```python
from build123d import *

# Parameters (mm, degrees)
BASE_PLATE_DEPTH       = 1
RIM_WALL_DEPTH         = 2
SIDE_GROOVE_A_SKETCH_W = 1
SIDE_GROOVE_A_SKETCH_H = 1
SIDE_GROOVE_A_DEPTH    = 40
SIDE_GROOVE_B_SKETCH_W = 1
SIDE_GROOVE_B_SKETCH_H = 1
SIDE_GROOVE_B_DEPTH    = 40


with BuildPart() as part:
    # Base Plate Sketch → Base Plate (new body)
    with BuildSketch(Plane(origin=(0, 0, 0), x_dir=(1, 0, 0), z_dir=(0, 1, 0))):
        with BuildLine():
            Line((-10.246950766, 12), (10.246950766, 12))
            ThreePointArc((10.246950766, 12), (12.001066805, 11.594868137), (13.399858694, 10.461538462))
            ThreePointArc((13.399858694, 10.461538462), (17, 0), (13.399858694, -10.461538462))
            ThreePointArc((13.399858694, -10.461538462), (12.001066805, -11.594868137), (10.246950766, -12))
            Line((10.246950766, -12), (-10.246950766, -12))
            ThreePointArc((-10.246950766, -12), (-12.001066805, -11.594868137), (-13.399858694, -10.461538462))
            ThreePointArc((-13.399858694, -10.461538462), (-17, 0), (-13.399858694, 10.461538462))
            ThreePointArc((-13.399858694, 10.461538462), (-12.001066805, 11.594868137), (-10.246950766, 12))
        make_face()
    extrude(amount=BASE_PLATE_DEPTH)

    # Rim Wall Sketch → Rim Wall (add)
    with BuildSketch(Plane(origin=(0, 1, 0), x_dir=(1, 0, 0), z_dir=(0, 1, 0))):
        with BuildLine():
            Line((10.246950766, -10), (-10.246950766, -10))
            ThreePointArc((-10.246950766, -10), (-11.124008785, -9.797434069), (-11.82340473, -9.230769231))
            ThreePointArc((-11.82340473, -9.230769231), (-15, 0), (-11.82340473, 9.230769231))
            ThreePointArc((-11.82340473, 9.230769231), (-11.124008785, 9.797434069), (-10.246950766, 10))
            Line((-10.246950766, 10), (10.246950766, 10))
            Line((10.246950766, 10), (13.747727085, 10))
            ThreePointArc((13.747727085, 10), (13.575754412, 10.232247659), (13.399858694, 10.461538462))
            ThreePointArc((13.399858694, 10.461538462), (12.001066805, 11.594868137), (10.246950766, 12))
            Line((10.246950766, 12), (-10.246950766, 12))
            ThreePointArc((-10.246950766, 12), (-12.001066805, 11.594868137), (-13.399858694, 10.461538462))
            ThreePointArc((-13.399858694, 10.461538462), (-17, 0), (-13.399858694, -10.461538462))
            ThreePointArc((-13.399858694, -10.461538462), (-12.001066805, -11.594868137), (-10.246950766, -12))
            Line((-10.246950766, -12), (10.246950766, -12))
            ThreePointArc((10.246950766, -12), (12.001066805, -11.594868137), (13.399858694, -10.461538462))
            ThreePointArc((13.399858694, -10.461538462), (13.575754412, -10.232247659), (13.747727085, -10))
            Line((13.747727085, -10), (10.246950766, -10))
        make_face()
    extrude(amount=RIM_WALL_DEPTH)

    # Side Groove A Sketch → Side Groove A (cut)
    with BuildSketch(Plane(origin=(30, 0, 0), x_dir=(0, 0, -1), z_dir=(1, 0, 0))):
        with Locations((-10.5, 1.5)):
            Rectangle(SIDE_GROOVE_A_SKETCH_W, SIDE_GROOVE_A_SKETCH_H)
    extrude(amount=-SIDE_GROOVE_A_DEPTH, mode=Mode.SUBTRACT)

    # Side Groove B Sketch → Side Groove B (cut)
    with BuildSketch(Plane(origin=(30, 0, 0), x_dir=(0, 0, -1), z_dir=(1, 0, 0))):
        with Locations((10.5, 1.5)):
            Rectangle(SIDE_GROOVE_B_SKETCH_W, SIDE_GROOVE_B_SKETCH_H)
    extrude(amount=-SIDE_GROOVE_B_DEPTH, mode=Mode.SUBTRACT)


solid = part.part
```
Work out the finished part from the listing and answer in its coordinate system (mm). A direction names the side the tool comes from. Round coordinates to 2 decimals unless told otherwise and drop trailing zeros. Write each loop counter-clockwise with the first axis right and the second up, starting at its lowest first coordinate (ties: lowest second). Pieces come first, ordered by that corner, then holes.
1) A cutting plane is placed at D-D on z = -4.5. Determine the outline of the cut face in (x, y).
2) Which of the six approach directions +Z, -Z, +X, -X, +Y, -Y give full straight-line access (tool end or side, diameter ignored) to faces 1 (the face through (2, 2, 10.5)), 2 (the face through (-11.14, 1.99, -9.79)), 3 (the face through (0, 1, -12))?
3) Consider probe 1 along Z at (x, y) = (0, 1.5); probe 2 along Z at (x, y) = (9, 2.1); probe 3 along Y at (x, z) = (6, 10.75). Determine where each line is inside the solid, lowest interval first.
4) A cutting plane is placed at B-B on x = 5.5. Determine the outline of the cut face in (y, z), and give its area (3 significant figures).
5) Flat-ended cylindrical pins translate along their axes: P1, Ø1, axis at y = 1, z = -4.5, coming from the -X side; P2, Ø2, axis at x = -12.5, z = 2.5, coming from the -Y side; P3, Ø3, axis at x = -10, z = -5.5, coming from the +Y side; P4, Ø0.8, axis at y = 1.5, z = 10.5, coming from the +X side. Find the tip coordinate at first contact, or state that the pin passes through.
6) A cutting plane is placed at C-C on z = -1.25. Determine the outline of the cut face in (x, y), and give its area (3 significant figures).
7) Determine the mould class of faces 4 (the face through (-15.4, 3, 0.8)), 5 (the face through (1.6, 1.5, -11)), 6 (the face through (1.6, 2.7, -10)) for opening direction Y: pulls with the +Y half, pulls with the -Y half, needs draft (parallel to the pull), parting line crosses it, or undercut.
8) A cutting plane is placed at A-A on y = 2.55. Determine the outline of the cut face in (x, z).
Entries:
1. outline: (-16.39, 0) - (16.39, 0) - (16.39, 1) - (-14.31, 1) - (-14.31, 3) - (-16.39, 3) - close
2. face 1: +X
2. face 2: +X, +Y
2. face 3: -Z, +X, -X, +Y, -Y
3. probe 1: z = -12 to -11, 11 to 12
3. probe 2: z = -12 to -10, 10 to 12
3. probe 3: y = 0 to 1, 2 to 3
4. outline: (0, -12) - (3, -12) - (3, -10) - (2, -10) - (2, -11) - (1, -11) - (1, 11) - (2, 11) - (2, 10) - (3, 10) - (3, 12) - (0, 12) - close
4. area: 30.0 mm2
5. P1: stops at x = -16.52
5. P2: stops at y = 0
5. P3: stops at y = 1
5. P4: stops at x = -10
6. outline: (-16.95, 0) - (16.95, 0) - (16.95, 1) - (-14.95, 1) - (-14.95, 3) - (-16.95, 3) - close
6. area: 37.9 mm2
7. face 4: pulls with the +Y half
7. face 5: undercut
7. face 6: needs draft
8. outline: (-13.4, -10.46) arc R4 ccw to (-10.25, -12) - (10.25, -12) arc R4 ccw to (13.4, -10.46) arc R17 ccw to (13.75, -10) - (-10.25, -10) arc R2 cw to (-11.82, -9.23) arc R15 cw to (-11.82, 9.23) arc R2 cw to (-10.25, 10) - (13.75, 10) arc R17 ccw to (13.4, 10.46) arc R4 ccw to (10.25, 12) - (-10.25, 12) arc R4 ccw to (-13.4, 10.46) arc R17 ccw to start
